from build123d import *


with BuildPart() as part:
    # 草图3 → 旋转19 (revolve)
    with BuildSketch(Plane.XY, mode=Mode.PRIVATE) as revolve_19_sk:
        Polygon((0, 10.070696149), (3.5, 10.070696149), (3.5, 5.070696149), (4.5, 5.070696149), (4.5, 1.070696149), (3.5, 1.070696149), (3.5, -8.929303851), (1.5, -8.929303851), (1.5, -17.929303851), (0, -17.929303851), align=None)
    revolve(revolve_19_sk.sketch.rotate(Axis((0, 0, 0), (0, 1, 0)), 90), axis=Axis((0, 0, 0), (0, 1, 0)))


solid = part.part
Design review of the part built by this model. Coordinates are the model's own, in mm. A direction names the side the tool comes from. Give positions to 0.01 mm unless a question says otherwise; leave off trailing zeros. Loops run counter-clockwise (first coordinate to the right, second up) from the corner with the lowest first, then second, coordinate; pieces in that order, holes last. Notation, with made-up numbers: M -34.75,-9 L 19.25,-9 A19 cw 19.25,2 Z; hole C 70.25,-23.5 d8. An arc over 180 degrees is marked long. Answer as a JSON object with one key per item and string values.
Item 1: We need section A-A (x = 0). State the section outline as (y, z) points.
Output values:
{"outline": "M -17.93,-1.5 L -8.93,-1.5 L -8.93,-3.5 L 1.07,-3.5 L 1.07,-4.5 L 5.07,-4.5 L 5.07,-3.5 L 10.07,-3.5 L 10.07,3.5 L 5.07,3.5 L 5.07,4.5 L 1.07,4.5 L 1.07,3.5 L -8.93,3.5 L -8.93,1.5 L -17.93,1.5 Z"}
Item 2: For P1, Ø1, axis at x = 1.5, z = 2, coming from the -Y side; P2, Ø2, axis at y = -11, z = 2, coming from the -X side; P3, Ø2, axis at x = -1.5, y = -10, coming from the -Z side, all flat-tipped, find the tip position at first contact; note any pin that passes through.
Output values:
{"P1": "stops at y = -8.93", "P2": "stops at x = -1.12", "P3": "stops at z = -1.41"}
Item 3: We need section B-B (z = 0). State the section outline as (x, y) points.
Output values:
{"outline": "M -4.5,1.07 L -3.5,1.07 L -3.5,-8.93 L -1.5,-8.93 L -1.5,-17.93 L 1.5,-17.93 L 1.5,-8.93 L 3.5,-8.93 L 3.5,1.07 L 4.5,1.07 L 4.5,5.07 L 3.5,5.07 L 3.5,10.07 L -3.5,10.07 L -3.5,5.07 L -4.5,5.07 Z"}
Item 4: We need section C-C (y = 6). State the section outline as (x, z) points.
Output values:
{"outline": "C 0,0 d7"}
Item 5: Wall thickness on line 1 along Y through (x, z) = (-1, 2); line 2 along Y through (x, z) = (-3.25, -2.75); line 3 along X through (y, z) = (-7.5, 0): over which ranges is each line inside the solid? List them lowest first.
Output values:
{"line 1": "y = -8.93 to 10.07", "line 2": "y = 1.07 to 5.07", "line 3": "x = -3.5 to 3.5"}
Item 6: Machinability: for faces 1 (the face through (3.105, 7.536, -1.615)), 2 (the face through (0, 10.071, 0)), 3 (the face through (3.105, -3.999, -1.615)), which of the approach directions +Z, -Z, +X, -X, +Y, -Y give a long, thin tool a straight path to every point of the face, cutting with its end or side? Answer none if there is none.
Output values:
{"face 1": "+Y", "face 2": "+Z, -Z, +X, -X, +Y", "face 3": "-Y"}
Item 7: We need section D-D (x = -2.75). State the section outline as (y, z) points.
Output values:
{"outline": "M -8.93,-2.17 L 1.07,-2.17 L 1.07,-3.56 L 5.07,-3.56 L 5.07,-2.17 L 10.07,-2.17 L 10.07,2.17 L 5.07,2.17 L 5.07,3.56 L 1.07,3.56 L 1.07,2.17 L -8.93,2.17 Z"}
